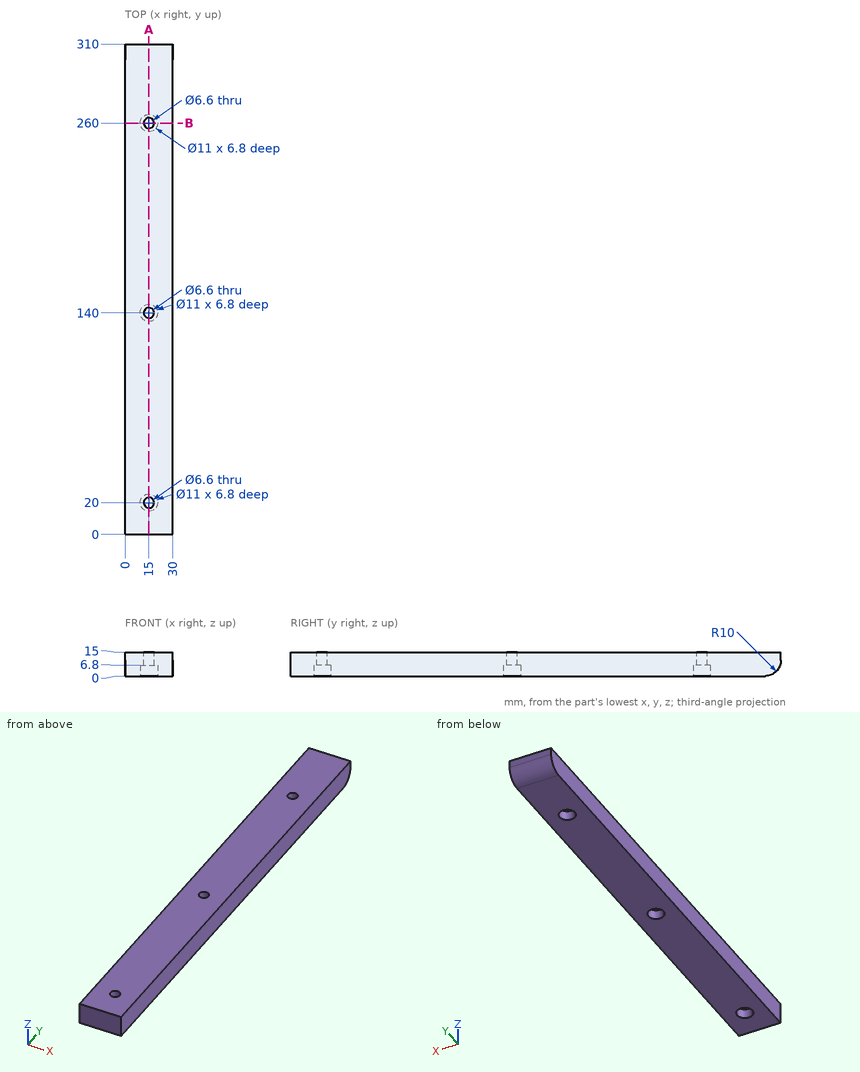
Study the drawing (mm; zero at the part's minimum x, y, z) and answer. Give positions to 0.01 mm unless a question says otherwise; leave off trailing zeros. Write each loop counter-clockwise with the first axis right and the second up, starting at its lowest first coordinate (ties: lowest second). Pieces come first, ordered by that corner, then holes. Notation, with made-up numbers: (-21.75, 58.5) -> (15.25, 58.5) arc R21 cw to (15.25, 90.5) -> close; hole circle Ø9 at (62.5, 71.5). An arc over 180 degrees is marked (long way). Write item = value, one per line. Start each with the question number.
1) The part is cut by section B-B, the plane y = 260. Determine the outline of the cut face in (x, z), and give its area (3 significant figures).
2) The part is cut by section A-A, the plane x = 15. Count the separate pieces of the cut face and the enclosed holes in it, and give its area (3 significant figures).
3) This flat-tipped pin is pushed along its axis until it touches: pin 1 (3.5 mm diameter, centred on x = 17.5, y = 138.5, fed in from -Z). Where does it stop, or does it pass through?
4) Straight lines are drawn through the part: line 1 along X through (y, z) = (20, 9.75); line 2 along Y through (x, z) = (15, 13); line 3 along Y through (x, z) = (18.75, 4.75). For each, find the intervals that lie inside material, in ascending order.
Solutions:
q1.outline = (0, 0) -> (9.5, 0) -> (9.5, 6.8) -> (11.7, 6.8) -> (11.7, 15) -> (0, 15) -> close; (18.3, 6.8) -> (20.5, 6.8) -> (20.5, 0) -> (30, 0) -> (30, 15) -> (18.3, 15) -> close
q1.area = 321 mm²
q2.separate_pieces = 4
q2.enclosed_holes = 0
q2.area = 4,240 mm²
q3.pin_1 = 6.8
q4.line_1 = 0 to 11.7, 18.3 to 30
q4.line_2 = 0 to 16.7, 23.3 to 136.7, 143.3 to 256.7, 263.3 to 310
q4.line_3 = 0 to 15.98, 24.02 to 135.98, 144.02 to 255.98, 264.02 to 308.51
